```python
from build123d import *

# Parameters (mm, degrees)
BOSS_EXTRUDE1_DEPTH = 10


with BuildPart() as part:
    # Sketch1 → Boss-Extrude1 (new body)
    with BuildSketch(Plane(origin=(0, 0, 0), x_dir=(0, 0, -1), z_dir=(1, 0, 0))):
        with BuildLine():
            Line((0, 145), (0, 344))
            Line((0, 344), (-8.216588633, 348.300204281))
            Line((-8.216588633, 348.300204281), (-222, 200))
            Line((-222, 200), (-178.231456798, 184.258681831))
            ThreePointArc((-178.231456798, 184.258681831), (-168.638904926, 176.941636961), (-165, 165.43883))
            Line((-165, 165.43883), (-165, 10))
            Line((-165, 10), (-157.488351016, 6.601146077))
            Line((-157.488351016, 6.601146077), (0, 145))
        make_face()
    extrude(amount=BOSS_EXTRUDE1_DEPTH)


solid = part.part
```
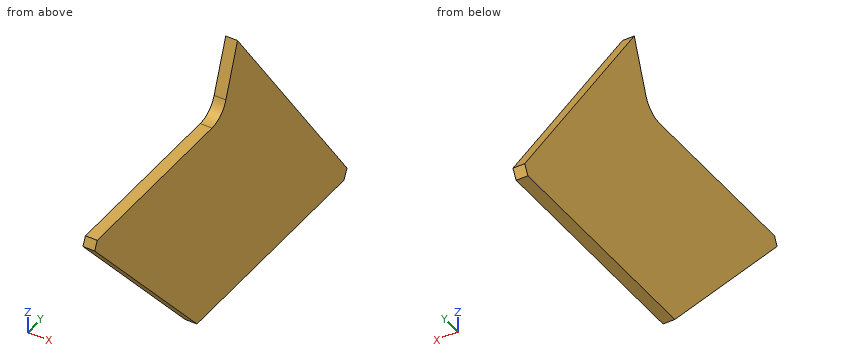
Model file for the job. Use its own axes, mm. Coordinates: 2 decimals unless noted, no trailing zeros. Order: outer loops, then holes, each group sorted by start corner. A loop starts at its lowest first (then second) coordinate and runs counter-clockwise, first axis right, second up. Notation, with made-up numbers: M -39,52.5 L -24,52.5 A34 cw -24,82.5 Z; hole C 41,53 d10. An arc over 180 degrees is marked long. Answer as CSV lines item,"result".
(1) Band-saw the part on B-B, the plane y = 156. List the corners of the cut face in (x, z).
Geometry says:
outline,"M 0,0 L 10,0 L 10,165 L 0,165 Z"
(2) Band-saw the part on C-C, the plane z = 79.5. List the corners of the cut face in (x, y).
Geometry says:
outline,"M 0,75.14 L 10,75.14 L 10,298.85 L 0,298.85 Z"
(3) Flat gauge pins, fed straight in: pin 1 (5 mm diameter, centred on x = 3, z = 134.5, fed in from -Y); pin 2 (1.5 mm diameter, centred on x = 8, z = 198.5, fed in from +Y); pin 3 (1.5 mm diameter, centred on x = 4.5, z = 162, fed in from -Y). Where does each tip first touch, or does it go through?
Geometry says:
pin 1,"stops at y = 24.61"
pin 2,"stops at y = 216.82"
pin 3,"stops at y = 8.3"
(4) Wall check: line 1 along Z through (x, y) = (1.75, 145); line 2 along Z through (x, y) = (5.75, 179); line 3 along Y through (x, z) = (3.75, 171). Give the ranges that are in metal, low to high.
Geometry says:
line 1,"z = 0 to 165"
line 2,"z = 0 to 170.3"
line 3,"y = 179.72 to 235.38"
(5) Band-saw the part on A-A, the plane x = 2.25. List the corners of the cut face in (y, z), then the cut area to 3 significant figures.
Geometry says:
outline,"M 6.6,157.49 L 145,0 L 344,0 L 348.3,8.22 L 200,222 L 184.26,178.23 A20 cw 165.44,165 L 10,165 Z"
area,"38,700 mm2"
